```python
from build123d import *

# Parameters (mm, degrees)
SKETCH1_R               = 24
BOSS_EXTRUDE1_DEPTH     = 20
CUT_EXTRUDE2_DEPTH      = 30
CUT_EXTRUDE2_DEPTH_BACK = 30
SKETCH3_R               = 3
SKETCH4_R               = 16
BOSS_EXTRUDE2_DEPTH     = 10
SKETCH5_R               = 10.5
CUT_EXTRUDE3_DEPTH      = 30
CHAMFER1_SIZE           = 1
CHAMFER2_SIZE           = 1


with BuildPart() as part:
    # Sketch1 → Boss-Extrude1 (new body)
    with BuildSketch(Plane(origin=(0, 0, 0), x_dir=(1, 0, 0), z_dir=(0, 1, 0))):
        with Locations(Location((0, 0, 0), (0, 0, 270))):
            Circle(SKETCH1_R)
    extrude(amount=BOSS_EXTRUDE1_DEPTH)

    # Sketch3 → Cut-Extrude2 (cut, two sides: drawn at the far end of the back side and taken through both)
    with BuildSketch(Plane(origin=(0, 0, 0), x_dir=(0, 0, -1), z_dir=(1, 0, 0)).offset(-CUT_EXTRUDE2_DEPTH_BACK)):
        with Locations(Location((0, 10, 0), (0, 0, 180))):
            Circle(SKETCH3_R)
    extrude(amount=CUT_EXTRUDE2_DEPTH + CUT_EXTRUDE2_DEPTH_BACK, mode=Mode.SUBTRACT)

    # Sketch4 → Boss-Extrude2 (add)
    with BuildSketch(Plane(origin=(0, 20, 0), x_dir=(1, 0, 0), z_dir=(0, 1, 0))):
        with Locations(Location((0, 0, 0), (0, 0, 270))):
            Circle(SKETCH4_R)
    extrude(amount=BOSS_EXTRUDE2_DEPTH)

    # Sketch5 → Cut-Extrude3 (cut)
    with BuildSketch(Plane(origin=(0, 30, 0), x_dir=(1, 0, 0), z_dir=(0, 1, 0))):
        with Locations(Location((0, 0, 0), (0, 0, 270))):
            Circle(SKETCH5_R)
    extrude(amount=-CUT_EXTRUDE3_DEPTH, mode=Mode.SUBTRACT)

    # Chamfer1
    chamfer1_edges = [part.edges().sort_by_distance(p)[0] for p in [
        (0, 20, -16),
        (0, 30, -16),
        (0, 0, -10.5),
        (0, 0, -24),
        (0, 20, -24),
    ]]
    chamfer(chamfer1_edges, length=CHAMFER1_SIZE)

    # Chamfer2
    chamfer2_edges = [part.edges().sort_by_distance(p)[0] for p in [
        (0, 30, -10.5),
    ]]
    chamfer(chamfer2_edges, length=CHAMFER2_SIZE)


solid = part.part
```
Design review of the part built by this model. Coordinates are the model's own, in mm. A direction names the side the tool comes from. Coordinates: 2 decimals unless noted, no trailing zeros. Order: outer loops, then holes, each group sorted by start corner. A loop starts at its lowest first (then second) coordinate and runs counter-clockwise, first axis right, second up. Notation, with made-up numbers: (50, -8.5) - (82, -8.5) arc R23 cw to (82, 25.5) - close; hole circle Ø2 at (-14.75, -9). An arc over 180 degrees is marked (long way). Answer in a Markdown table with one row per item.
(1) Consider section B-B on z = 0. Give the number of separate pieces and of enclosed holes in the cut face, plus the area to 3 significant figures.
Checked values:
| item | result |
|---|---|
| separate pieces | 4 |
| enclosed holes | 0 |
| area | 484 mm^2 |
(2) Consider section C-C on y = 2. State the section outline as (x, z) points.
Checked values:
| item | result |
|---|---|
| outline | circle Ø48 at (0, 0); hole circle Ø21 at (0, 0) |
(3) Consider section D-D on y = 10. State the section outline as (x, z) points.
Checked values:
| item | result |
|---|---|
| outline | (-23.81, -3) arc R24 ccw to (23.81, -3) - (10.06, -3) arc R10.5 cw to (-10.06, -3) - close; (-23.81, 3) - (-10.06, 3) arc R10.5 cw to (10.06, 3) - (23.81, 3) arc R24 ccw to start |
(4) The part is to be moulded in two halves that separate along X. For faces 3 (the cylindrical face through (-9.315, 15.196, 4.845)), 4 (the flat face through (-9, 30, 8)), 5 (the cylindrical face through (7.21, 9.87, 22.89)), say which applies: released by +X, released by -X, zero draft, split by the parting line, or undercut.
Checked values:
| item | result |
|---|---|
| face 3 | undercut |
| face 4 | zero draft |
| face 5 | split by the parting line |
(5) For faces 1 (the cylindrical face through (-15.62, 24.94, -3.47)), 2 (the flat face through (11, 0, 5)), list the 3-axis set-ups (+Z, -Z, +X, -X, +Y, -Y) from which the entire face can be reached by the end or side of a thin tool; tool diameter is ignored.
Checked values:
| item | result |
|---|---|
| face 1 | +Y |
| face 2 | +Z, -Z, +X, -X, -Y |
(6) Wall thickness on line 1 along X through (y, z) = (16.75, 0.5); line 2 along Y through (x, z) = (-17, 5); line 3 along Z through (x, y) = (16.75, 10): over which ranges is each line inside the solid? List them lowest first. Write a range as from..to.
Checked values:
| item | result |
|---|---|
| line 1 | -23.99..-10.49, 10.49..23.99 |
| line 2 | 0..20 |
| line 3 | -17.19..-3, 3..17.19 |
(7) Clearance check with flat-ended pins moving along their axes: pin 1 (2 mm diameter, centred on x = -8.5, y = 24, fed in from -Z); pin 2 (5 mm diameter, centred on x = 9, y = 16.5, fed in from -Z); pin 3 (1 mm diameter, centred on x = -10.5, y = 11, fed in from -Z). State where each tip first meets the part, or that it passes through.
Checked values:
| item | result |
|---|---|
| pin 1 | z = -14.13 |
| pin 2 | z = -23.1 |
| pin 3 | z = -21.82 |
(8) Consider section A-A on x = 0. State the section outline as (y, z) points, plus the area to 3 significant figures.
Checked values:
| item | result |
|---|---|
| outline | (0, -23) - (1, -24) - (19, -24) - (20, -23) - (20, -17) - (21, -16) - (29, -16) - (30, -15) - (30, -11.5) - (29, -10.5) - (1, -10.5) - (0, -11.5) - close; (0, 11.5) - (1, 10.5) - (29, 10.5) - (30, 11.5) - (30, 15) - (29, 16) - (21, 16) - (20, 17) - (20, 23) - (19, 24) - (1, 24) - (0, 23) - close |
| area | 646 mm^2 |
